For this review, use the dimensioned drawing (mm, ordinates from the lowest corner) and the shaded views. A direction names the side the tool comes from. Coordinates: 2 decimals unless noted, no trailing zeros. Order: outer loops, then holes, each group sorted by start corner. A loop starts at its lowest first (then second) coordinate and runs counter-clockwise, first axis right, second up. Notation, with made-up numbers: M 35,75.25 L 70,75.25 A24 cw 70,110.25 Z; hole C -1,-7.5 d1. An arc over 180 degrees is marked long. One line per item, written item: value.
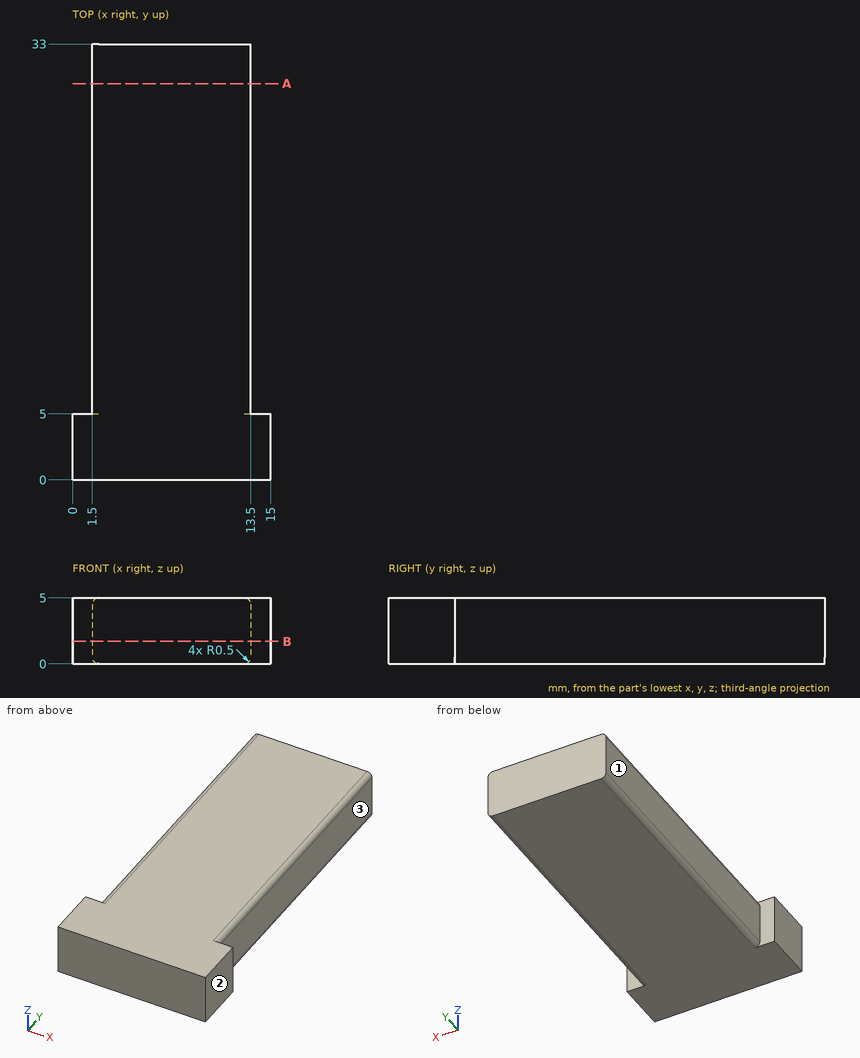
(1) We need section B-B, the plane z = 1.7. State the section outline as (x, y) points.
Geometry results:
outline: M 0,0 L 15,0 L 15,5 L 13.5,5 L 13.5,33 L 1.5,33 L 1.5,5 L 0,5 Z
(2) Insertion check: pin 1 Ø1.2 at (y, z) = (15.5, 2) entering from -X; pin 2 Ø2 at (y, z) = (15.5, 2.5) entering from +X; pin 3 Ø0.6 at (x, z) = (0.5, 3) entering from +Y. Each pin has a flat end and moves straight along its axis. Give the tip position at first contact, or say it passes through.
Geometry results:
pin 1: stops at x = 1.5
pin 2: stops at x = 13.5
pin 3: stops at y = 5
(3) For L1, parallel to X at y = 6, z = 2.25; L2, parallel to Y at x = 14, z = 2; L3, parallel to X at y = 30, z = 0.2, list the stretches that pass through material, from the lowest coordinate up.
Geometry results:
L1: x = 1.5 to 13.5
L2: y = 0 to 5
L3: x = 1.6 to 13.4
(4) Tool access review of the marked faces 1, 2 and 3: name each direction out of +Z, -Z, +X, -X, +Y, -Y from which nothing blocks a thin tool from reaching the whole face with its end or side.
Geometry results:
face 1: +Z, -Z, -X, +Y
face 2: +Z, -Z, +X, +Y, -Y
face 3: +Z, -Z, +X, +Y
(5) We need section A-A, the plane y = 30. State the section outline as (x, z) points, plus the area to 3 significant figures.
Geometry results:
outline: M 1.5,0.5 A0.5 ccw 2,0 L 13,0 A0.5 ccw 13.5,0.5 L 13.5,4.5 A0.5 ccw 13,5 L 2,5 A0.5 ccw 1.5,4.5 Z
area: 59.8 mm2
